The listing builds one solid part. Answer for the finished solid, in the listing's coordinates (mm). Face numbers are marked on the shaded views. Give positions to 0.01 mm unless a question says otherwise; leave off trailing zeros. Loops run counter-clockwise (first coordinate to the right, second up) from the corner with the lowest first, then second, coordinate; pieces in that order, holes last. Notation, with made-up numbers: (-14, 29) - (35, 29) arc R26 cw to (35, 64) - close; hole circle Ø4 at (30.5, -35.75). An arc over 180 degrees is marked (long way). One line per item, written item: value. Start each with the question number.
from build123d import *

# Parameters (mm, degrees)
BOSS_EXTRUDE1_DEPTH = 3


with BuildPart() as part:
    # Sketch1 → Boss-Extrude1 (new body)
    with BuildSketch(Plane.XY):
        with BuildLine():
            Line((0, 0), (5.5, 0))
            Line((5.5, 0), (5.5, 9.5))
            ThreePointArc((5.5, 9.5), (10, 14), (14.5, 9.5))
            Line((14.5, 9.5), (14.5, 0))
            Line((14.5, 0), (20.5, 0))
            Line((20.5, 0), (20.5, 9.5))
            ThreePointArc((20.5, 9.5), (25, 14), (29.5, 9.5))
            Line((29.5, 9.5), (29.5, 0))
            Line((29.5, 0), (35.5, 0))
            Line((35.5, 0), (35.5, 9.5))
            ThreePointArc((35.5, 9.5), (40, 14), (44.5, 9.5))
            Line((44.5, 9.5), (44.5, 0))
            Line((44.5, 0), (50, 0))
            Line((50, 0), (50, 19))
            Line((50, 19), (0, 19))
            Line((0, 19), (0, 0))
        make_face()
    extrude(amount=BOSS_EXTRUDE1_DEPTH)


solid = part.part
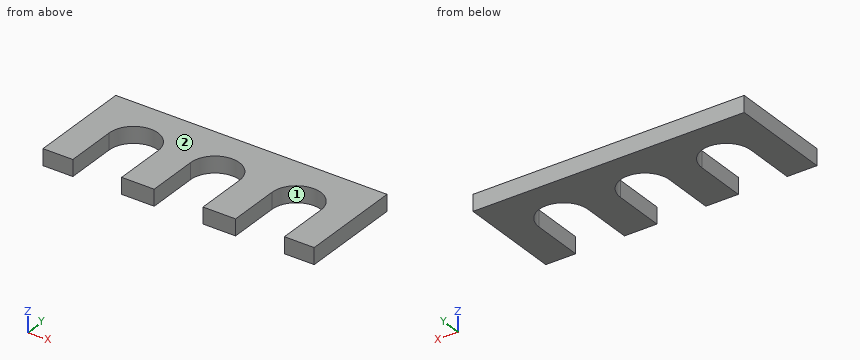
1. Determine the mould class of the marked faces 1 and 2 for opening direction X: released by +X, released by -X, zero draft, split by the parting line, or undercut.
2. A cutting plane is placed at D-D (x = 9.5). Determine the outline of the cut face in (y, z), plus the area to 3 significant figures.
3. A cutting plane is placed at A-A (y = 12.75). Determine the outline of the cut face in (x, z), plus the area to 3 significant figures.
4. A cutting plane is placed at C-C (x = 40). Determine the outline of the cut face in (y, z).
5. Find the intervals of material crossed by L1, parallel to X at y = 7, z = 1.6; L2, parallel to X at y = 11, z = 0.55; L3, parallel to Y at x = 24.5, z = 1.75, in increasing order. Write a range as [from, to].
6. A cutting plane is placed at B-B (z = 0.95). Determine the outline of the cut face in (x, y), plus the area to 3 significant figures.
Results below:
1. face 1: undercut
1. face 2: zero draft
2. outline: (13.97, 0) - (19, 0) - (19, 3) - (13.97, 3) - close
2. area: 15.1 mm^2
3. outline: (0, 0) - (6.89, 0) - (6.89, 3) - (0, 3) - close; (13.11, 0) - (21.89, 0) - (21.89, 3) - (13.11, 3) - close; (28.11, 0) - (36.89, 0) - (36.89, 3) - (28.11, 3) - close; (43.11, 0) - (50, 0) - (50, 3) - (43.11, 3) - close
3. area: 94.0 mm^2
4. outline: (14, 0) - (19, 0) - (19, 3) - (14, 3) - close
5. L1: x = [0, 5.5], [14.5, 20.5], [29.5, 35.5], [44.5, 50]
5. L2: x = [0, 5.76], [14.24, 20.76], [29.24, 35.76], [44.24, 50]
5. L3: y = [13.97, 19]
6. outline: (0, 0) - (5.5, 0) - (5.5, 9.5) arc R4.5 cw to (14.5, 9.5) - (14.5, 0) - (20.5, 0) - (20.5, 9.5) arc R4.5 cw to (29.5, 9.5) - (29.5, 0) - (35.5, 0) - (35.5, 9.5) arc R4.5 cw to (44.5, 9.5) - (44.5, 0) - (50, 0) - (50, 19) - (0, 19) - close
6. area: 598 mm^2
